CAD build for the part. Positions are in the model's coordinates, mm. A direction names the side the tool comes from. Give positions to 0.01 mm unless a question says otherwise; leave off trailing zeros. Loops run counter-clockwise (first coordinate to the right, second up) from the corner with the lowest first, then second, coordinate; pieces in that order, holes last. Notation, with made-up numbers: M 15.25,-17.75 L 42.25,-17.75 A32 cw 42.25,21.25 Z; hole C 65.5,27.5 d2. An arc over 180 degrees is marked long. One line per question, with ' | ' between items.
```python
from build123d import *

# Parameters (mm, degrees)
CUT_EXTRUDE_1_DEPTH = 1
CHAMFER_1_SIZE      = 0.6135


with BuildPart() as part:
    # 草图1 → 旋转1 (revolve)
    with BuildSketch(Plane(origin=(0, 0, 0), x_dir=(1, 0, 0), z_dir=(0, 1, 0))):
        Polygon((3, 12), (0, 12), (0, 0), (6, 0), (6, 0.5), (3, 3.3), align=None)
    revolve(axis=Axis((0, 0, -12), (0, 0, 1)))

    # 草图2 → 切除-拉伸1 (cut)
    with BuildSketch(Plane.XY):
        Polygon((1.5, -2.598076211), (3, 0), (1.5, 2.598076211), (-1.5, 2.598076211), (-3, 0), (-1.5, -2.598076211), align=None)
    extrude(amount=-CUT_EXTRUDE_1_DEPTH, mode=Mode.SUBTRACT)

    # 倒角1
    chamfer_1_edges = [part.edges().sort_by_distance(p)[0] for p in [
        (-3, 0, -12),
    ]]
    chamfer(chamfer_1_edges, length=CHAMFER_1_SIZE)


solid = part.part
```
Item 1: 3-axis set-ups, long thin cutter, end or side, ignore diameter. For faces 4 (the cylindrical face through (-3, 0, -7)), 5 (the flat face through (0, 0, -12)), 6 (the flat face through (0, 2.598, -0.5)): which of +Z, -Z, +X, -X, +Y, -Y reach the whole face in a straight line?
Conclusion:
face 4: -Z | face 5: -Z, +X, -X, +Y, -Y | face 6: +Z
Item 2: Saw through at A-A on x = 0. Give the cut face in (y, z), and give its area (3 significant figures).
Conclusion:
outline: M -6,-0.5 L -3,-3.3 L -3,-11.39 L -2.39,-12 L 2.39,-12 L 3,-11.39 L 3,-3.3 L 6,-0.5 L 6,0 L 2.6,0 L 2.6,-1 L -2.6,-1 L -2.6,0 L -6,0 Z | area: 77.8 mm²
Item 3: Saw through at C-C on z = -1.5. Give the cut face in (x, y), and give its area (3 significant figures).
Conclusion:
outline: C 0,0 d9.86 | area: 76.3 mm²
Item 4: Saw through at B-B on z = -10. Give the cut face in (x, y).
Conclusion:
outline: C 0,0 d6
Item 5: Mould opens along Y. For faces 1 (the flat face through (0, 3, 0)), 2 (the flat face through (-2.24, 1.32, -0.49)), 3 (the cylindrical face through (-5.994, 0.264, -0.254)) say: pulls with the +Y half, pulls with the -Y half, needs draft (parallel to the pull), parting line crosses it, or undercut.
Conclusion:
face 1: needs draft | face 2: undercut | face 3: parting line crosses it
Item 6: Drill centre lines: line 1 along Z through (x, y) = (1, -1); line 2 along Y through (x, z) = (-3.5, -2); line 3 along Y through (x, z) = (-2, -4.5). Where is each one in solid material? Low to high. Write a range as [from, to].
Conclusion:
line 1: [-12, -1] | line 2: [-2.65, 2.65] | line 3: [-2.24, 2.24]
Item 7: Drop flat-ended pins along their axis: P1, Ø2.5, axis at x = -0.5, y = 1, coming from the +Z side; P2, Ø3, axis at x = -0.5, y = 4, coming from the +Z side; P3, Ø5, axis at x = -3.5, z = -4, coming from the -Y side; P4, Ø6, axis at y = -0.5, z = -8, coming from the +X side. Give the stop position or say it passes through.
Conclusion:
P1: z = -1 | P2: z = 0 | P3: y = -3.99 | P4: x = 3
